Check sheet for the modelled part. Datum: model origin and axes. Units: mm. Give positions to 0.01 mm unless a question says otherwise; leave off trailing zeros. Order: outer loops, then holes, each group sorted by start corner. A loop starts at its lowest first (then second) coordinate and runs counter-clockwise, first axis right, second up. Notation, with made-up numbers: (29.5, -22.5) -> (51.5, -22.5) arc R16 ccw to (51.5, -12.5) -> close; hole circle Ø10 at (40, -26). An arc over 180 degrees is marked (long way). Answer in a Markdown table with one row per item. Add a question column.
(1) Thickness scan on L1, parallel to Y at x = 0, z = 21.5; L2, parallel to Y at x = 0, z = 19.75; L3, parallel to X at y = 143.5, z = 20.75. Record the ranges inside material, lowest first. Write a range as [from, to].
(2) Cross-section at B-B (y = -2). Record the cut outline in (x, z), then the cut area to 3 significant figures.
(3) Go/stop test with flat-tipped pins: pin 1 (8 mm diameter, centred on x = 0, y = 148, fed in from +Z); pin 2 (3 mm diameter, centred on x = -1, z = 14.5, fed in from +Y); pin 3 (7.5 mm diameter, centred on x = 0, y = 149.5, fed in from +Z); pin 4 (5 mm diameter, centred on x = -3.5, z = 20.5, fed in from +Y). Record where each tip stops, or that it passes through.
(4) Cross-section at C-C (y = 59). Record the cut outline in (x, z), then the cut area to 3 significant figures.
(5) Cross-section at D-D (y = 148). Record the cut outline in (x, z).
(6) Cross-section at A-A (x = 0). State how many separate pieces and enclosed holes the cut face has, then the cut area to 3 significant figures.
```python
from build123d import *

# Parameters (mm, degrees)
SKETCH1_W                                          = 40
SKETCH1_H                                          = 366
BOSS_EXTRUDE1_DEPTH                                = 25
SKETCH4_R                                          = 7.5
CUT_EXTRUDE1_DEPTH                                 = 2
HOLE_SIZE_BASED_ON_HEX_SOCKET_CAP_SCRE_D           = 9
HOLE_SIZE_BASED_ON_HEX_SOCKET_CAP_SCRE_CBORE_D     = 15
HOLE_SIZE_BASED_ON_HEX_SOCKET_CAP_SCRE_CBORE_DEPTH = 10
CUT_EXTRUDE4_DEPTH                                 = 15
CHAMFER4_SIZE                                      = 5
CUT_EXTRUDE5_DEPTH                                 = 189.981480574
FILLET3_R                                          = 15


with BuildPart() as part:
    # Sketch1 → Boss-Extrude1 (new body)
    with BuildSketch(Plane.XY):
        Rectangle(SKETCH1_W, SKETCH1_H)
    extrude(amount=BOSS_EXTRUDE1_DEPTH)

    # Sketch4 → Cut-Extrude1 (cut)
    with BuildSketch(Plane.XY.offset(25)):
        with Locations((0, -152)):
            Circle(SKETCH4_R)
        with Locations((0, -2)):
            Circle(SKETCH4_R)
        with Locations((0, 148)):
            Circle(SKETCH4_R)
    extrude(amount=-CUT_EXTRUDE1_DEPTH, mode=Mode.SUBTRACT)

    # Hole Size (based on) hex socket cap screw type 1 (through all)
    with Locations(Plane.XY.offset(23)):
        with Locations((0, -152), (0, -2), (0, 148)):
            CounterBoreHole(HOLE_SIZE_BASED_ON_HEX_SOCKET_CAP_SCRE_D / 2, HOLE_SIZE_BASED_ON_HEX_SOCKET_CAP_SCRE_CBORE_D / 2, HOLE_SIZE_BASED_ON_HEX_SOCKET_CAP_SCRE_CBORE_DEPTH)

    # Sketch13 → Cut-Extrude4 (cut)
    with BuildSketch(Plane(origin=(-32.686463761, 3.77430773, 18.871538651), x_dir=(0.46855304860894914, -0.22010109077968257, 0.855577904387937), z_dir=(-0.8617274844321422, 0.09950371902099794, 0.49751859510498975))):
        Polygon((-6.250003897, 80.225632862), (-22.8497284, 179.511998894), (-45.371671063, 174.403630071), align=None)
    cut_extrude4 = extrude(amount=CUT_EXTRUDE4_DEPTH, mode=Mode.SUBTRACT)

    # Mirror1: Cut-Extrude4 across plane
    add(cut_extrude4.mirror(Plane.ZY), mode=Mode.SUBTRACT)

    # Chamfer4
    chamfer4_edges = [part.edges().sort_by_distance(p)[0] for p in [
        (-20, -50, 25),
        (20, -50, 25),
    ]]
    chamfer(chamfer4_edges, length=CHAMFER4_SIZE)

    # Sketch14 → Cut-Extrude5 (cut, through all)
    with BuildSketch(Plane.ZY.offset(20)):
        Polygon((5, 183), (25, 163), (25, 183), align=None)
    extrude(amount=-CUT_EXTRUDE5_DEPTH, mode=Mode.SUBTRACT)

    # Fillet3
    fillet3_edges = [part.edges().sort_by_distance(p)[0] for p in [
        (0, 163, 25),
    ]]
    fillet(fillet3_edges, radius=FILLET3_R)


solid = part.part
```
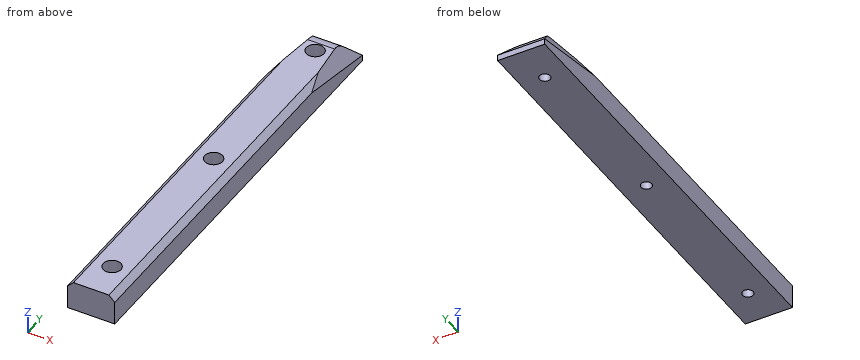
Answer below:
| question | item | result |
|---|---|---|
| 1 | L1 | y = [-183, -159.5], [-144.5, -9.5], [5.5, 140.5], [155.5, 166.42] |
| 1 | L2 | y = [-183, -159.5], [-144.5, -9.5], [5.5, 140.5], [155.5, 168.25] |
| 1 | L3 | x = [-15.47, -6], [6, 15.47] |
| 2 | outline | (-20, 0) -> (-4.5, 0) -> (-4.5, 13) -> (-7.5, 13) -> (-7.5, 25) -> (-15, 25) -> (-20, 20) -> close; (4.5, 0) -> (20, 0) -> (20, 20) -> (15, 25) -> (7.5, 25) -> (7.5, 13) -> (4.5, 13) -> close |
| 2 | area | 678 mm² |
| 3 | pin 1 | passes through |
| 3 | pin 2 | stops at y = 175 |
| 3 | pin 3 | stops at z = 13 |
| 3 | pin 4 | stops at y = 170 |
| 4 | outline | (-20, 0) -> (20, 0) -> (20, 20) -> (15, 25) -> (-15, 25) -> (-20, 20) -> close |
| 4 | area | 975 mm² |
| 5 | outline | (-20, 0) -> (-4.5, 0) -> (-4.5, 13) -> (-7.5, 13) -> (-7.5, 25) -> (-12.49, 25) -> (-20, 12) -> close; (4.5, 0) -> (20, 0) -> (20, 12) -> (12.49, 25) -> (7.5, 25) -> (7.5, 13) -> (4.5, 13) -> close |
| 6 | separate pieces | 4 |
| 6 | enclosed holes | 0 |
| 6 | area | 8,050 mm² |
